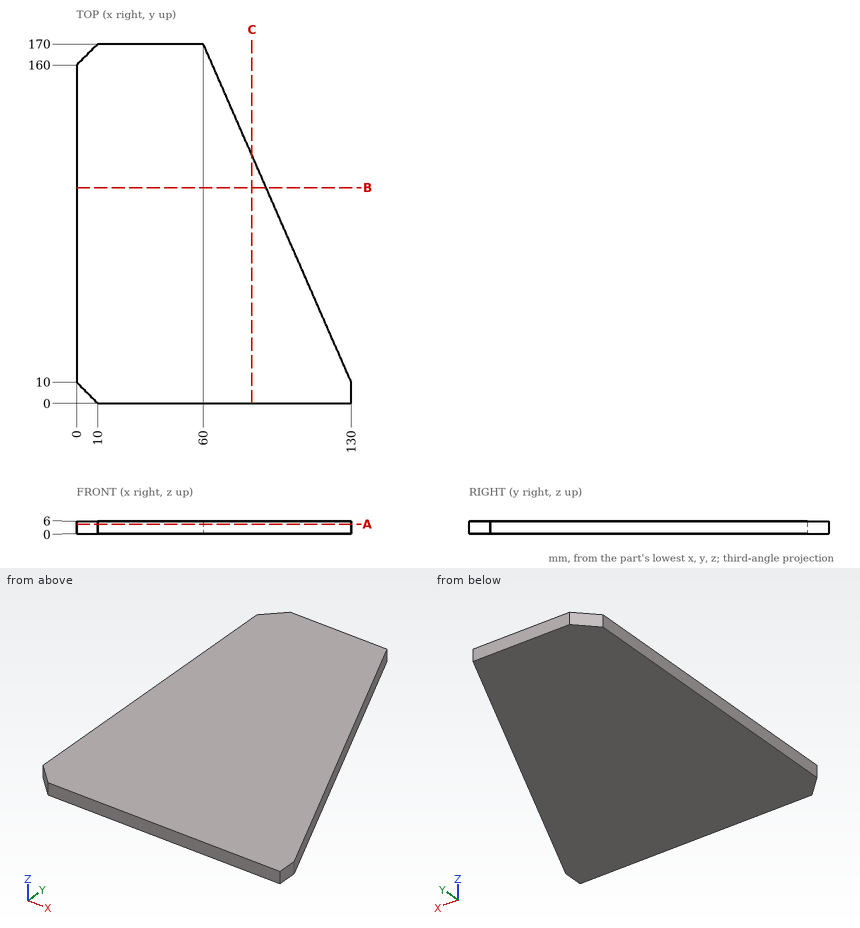
The drawing under review shows one solid part. Ordinate dimensions are in mm from its lowest x, y, z. Round coordinates to 2 decimals unless told otherwise and drop trailing zeros. Loops run counter-clockwise (first coordinate to the right, second up) from the corner with the lowest first, then second, coordinate; pieces in that order, holes last. Notation, with made-up numbers: (-37.75, -19) - (11.25, -19) arc R22 cw to (11.25, 8) - close; hole circle Ø5 at (83.25, -34.5). An arc over 180 degrees is marked (long way). One line per question, with ' | ' between items.
Q1. For pin 1 (3 mm diameter, centred on x = 70, z = 5, fed in from +Y), flat-tipped, find the tip position at first contact; note if it passes through.
Taken from the geometry:
pin 1: stops at y = 150.57
Q2. Take a section at B-B (y = 102). Give the boundary of the cut face in (x, z).
Taken from the geometry:
outline: (0, 0) - (89.75, 0) - (89.75, 6) - (0, 6) - close
Q3. Take a section at C-C (x = 83). Give the boundary of the cut face in (y, z), and give its area (3 significant figures).
Taken from the geometry:
outline: (0, 0) - (117.43, 0) - (117.43, 6) - (0, 6) - close | area: 705 mm²
Q4. Take a section at A-A (z = 4.65). Give the boundary of the cut face in (x, y), and give its area (3 significant figures).
Taken from the geometry:
outline: (0, 10) - (10, 0) - (130, 0) - (130, 10) - (60, 170) - (10, 170) - (0, 160) - close | area: 16,400 mm²
Q5. For line 1 along Y through (x, z) = (62.5, 2.9); line 2 along X through (y, z) = (42.5, 3.6); line 3 along X through (y, z) = (74.5, 0.75), list the stretches that pass through material, from the lowest coordinate up. Write a range as [from, to].
Taken from the geometry:
line 1: y = [0, 164.29] | line 2: x = [0, 115.78] | line 3: x = [0, 101.78]
